Drawing for the job (mm, zero at the part's lowest x, y, z). A direction names the side the tool comes from. Give positions to 0.01 mm unless a question says otherwise; leave off trailing zeros. Loops run counter-clockwise (first coordinate to the right, second up) from the corner with the lowest first, then second, coordinate; pieces in that order, holes last. Notation, with made-up numbers: (33.5, 61.25) -> (52.5, 61.25) arc R29 ccw to (52.5, 90.25) -> close; hole circle Ø9 at (-4, 23.25). An arc over 180 degrees is marked (long way). Answer in a Markdown table with one row per item. Add a question column.
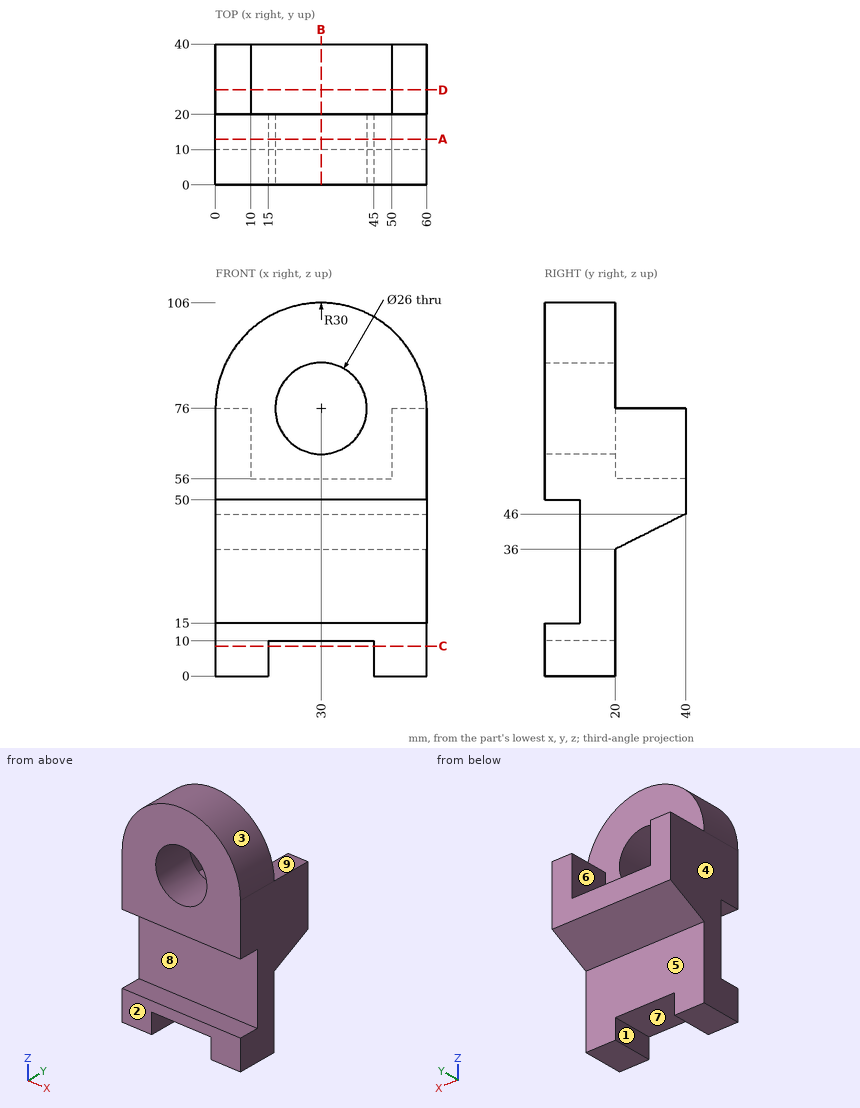
(1) Saw through at C-C, the plane z = 8.5. List the corners of the cut face in (x, y).
(2) Two-plate mould, pull along X, no slides. Class the marked faces 1, 2, 3 and 4: released by +X, released by -X, zero draft, split by the parting line, or undercut.
(3) Wall check: line 1 along Z through (x, y) = (30, 6); line 2 along X through (y, z) = (14, 76); line 3 along Z through (x, y) = (37.5, 2.5). Give the ranges that are in metal, low to high. Write a range as from..to.
(4) 3-axis set-ups, long thin cutter, end or side, ignore diameter. For the marked faces 5, 6, 7, 8 and 9: which of +Z, -Z, +X, -X, +Y, -Y reach the whole face in a straight line?
(5) Flat gauge pins, fed straight in: pin 1 Ø3 at (y, z) = (13, 92.5) entering from -X; pin 2 Ø6 at (x, y) = (30.5, 11) entering from -Z; pin 3 Ø6 at (x, y) = (48.5, 29.5) entering from -Z. Where does each tip first touch, or does it go through?
(6) Saw through at A-A, the plane y = 13. List the corners of the cut face in (x, z).
(7) Saw through at B-B, the plane x = 30. List the corners of the cut face in (y, z).
(8) Saw through at D-D, the plane y = 27. List the corners of the cut face in (x, z), then the cut area to 3 significant figures.
Worked answers:
| question | item | result |
|---|---|---|
| 1 | outline | (0, 0) -> (15, 0) -> (15, 20) -> (0, 20) -> close; (45, 0) -> (60, 0) -> (60, 20) -> (45, 20) -> close |
| 2 | face 1 | undercut |
| 2 | face 2 | zero draft |
| 2 | face 3 | split by the parting line |
| 2 | face 4 | released by -X |
| 3 | line 1 | 10..15, 50..63, 89..106 |
| 3 | line 2 | 0..17, 43..60 |
| 3 | line 3 | 10..15, 50..65.38, 86.62..105.05 |
| 4 | face 5 | -Z, +X, -X, +Y |
| 4 | face 6 | +Z, +Y |
| 4 | face 7 | -Z, +Y, -Y |
| 4 | face 8 | +X, -X, -Y |
| 4 | face 9 | +Z, +X, -X, +Y |
| 5 | pin 1 | x = 4.02 |
| 5 | pin 2 | z = 10 |
| 5 | pin 3 | z = 39.25 |
| 6 | outline | (0, 0) -> (15, 0) -> (15, 10) -> (45, 10) -> (45, 0) -> (60, 0) -> (60, 76) arc R30 ccw to (0, 76) -> close; hole circle Ø26 at (30, 76) |
| 7 | outline | (0, 10) -> (20, 10) -> (20, 36) -> (40, 46) -> (40, 56) -> (20, 56) -> (20, 63) -> (0, 63) -> (0, 50) -> (10, 50) -> (10, 15) -> (0, 15) -> close; (0, 89) -> (20, 89) -> (20, 106) -> (0, 106) -> close |
| 8 | outline | (0, 39.5) -> (60, 39.5) -> (60, 76) -> (50, 76) -> (50, 56) -> (10, 56) -> (10, 76) -> (0, 76) -> close |
| 8 | area | 1,390 mm^2 |
